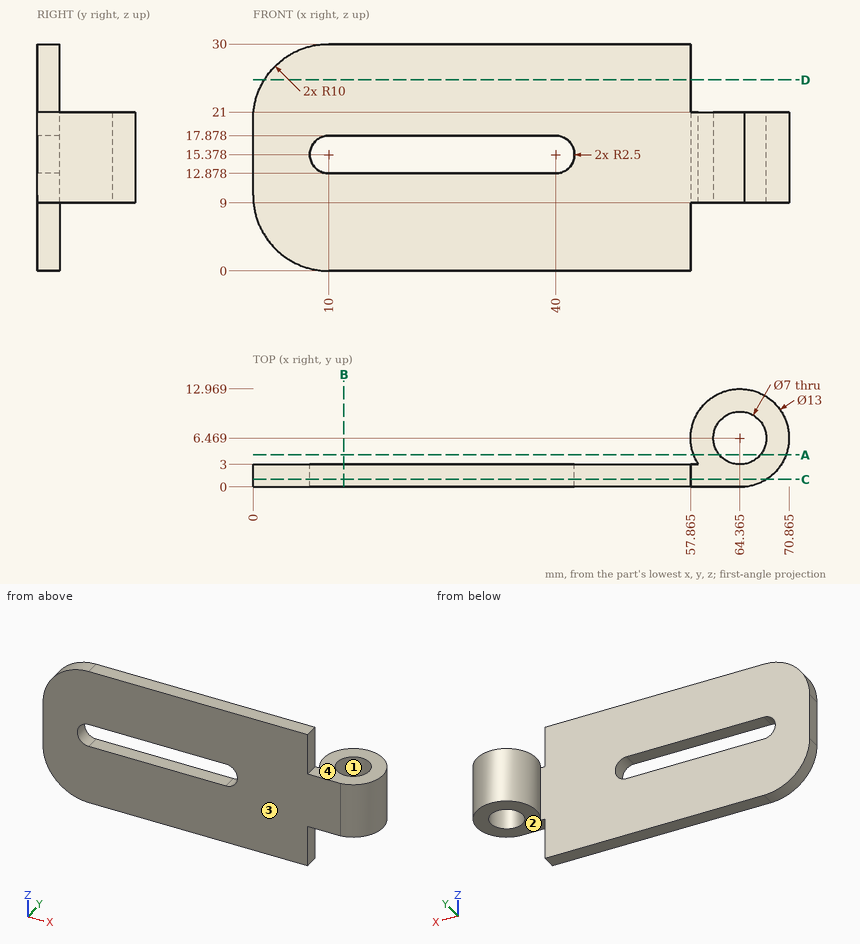
For this review, use the dimensioned drawing (mm, ordinates from the lowest corner) and the shaded views. A direction names the side the tool comes from. Round coordinates to 2 decimals unless told otherwise and drop trailing zeros. Loops run counter-clockwise (first coordinate to the right, second up) from the corner with the lowest first, then second, coordinate; pieces in that order, holes last. Notation, with made-up numbers: (62, 59.25) -> (120, 59.25) arc R25 cw to (120, 93.25) -> close; hole circle Ø8 at (3, 26.25). An arc over 180 degrees is marked (long way). Write item = value, one per line. Start each with the question number.
Item 1: To check wall thickness, follow L1, parallel to Z at x = 26, y = 2; L2, parallel to Y at x = 42, z = 12.5; L3, parallel to X at y = 7.25, z = 10.5 (1 decimal). State the ranges of each line that lie inside material, in increasing order.
Item 2: For the marked faces 3 and 4, list the 3-axis set-ups (+Z, -Z, +X, -X, +Y, -Y) from which the entire face can be reached by the end or side of a thin tool; tool diameter is ignored.
Item 3: Insertion check: pin 1 (2.5 mm diameter, centred on y = 1.5, z = 4, fed in from +X) (1 decimal); pin 2 (6.5 mm diameter, centred on x = 64.5, y = 5, fed in from +Z); pin 3 (6 mm diameter, centred on y = 4.5, z = 23.5, fed in from -X). Each pin has a flat end and moves straight along its axis. Give the tip position at first contact, or say it passes through.
Item 4: Take a section at A-A on y = 4.25. Give the boundary of the cut face in (x, z) (1 decimal).
Item 5: Mouldability with a two-part tool opening along X and no side actions: class the marked faces 1 and 2 as released by +X, released by -X, zero draft, split by the parting line, or undercut.
Item 6: Take a section at D-D on z = 25.25. Give the boundary of the cut face in (x, y) (1 decimal).
Item 7: Take a section at B-B on x = 12. Give the boundary of the cut face in (y, z).
Item 8: Take a section at C-C on y = 1. Give the boundary of the cut face in (x, z) (1 decimal), plus the area to 3 significant figures.
Result:
q1.L1 = 0 to 12.88, 17.88 to 30
q1.L2 = 0 to 3
q1.L3 = 57.9 to 61, 67.8 to 70.8
q2.face_3 = +Z, -Z, +X, -X, -Y
q2.face_4 = +Z, +X, +Y, -Y
q3.pin_1 = 57.9
q3.pin_2 = 21
q3.pin_3 = 0.04
q4.outline = (58.3, 9) -> (61.7, 9) -> (61.7, 21) -> (58.3, 21) -> close; (67.1, 9) -> (70.5, 9) -> (70.5, 21) -> (67.1, 21) -> close
q5.face_1 = undercut
q5.face_2 = zero draft
q6.outline = (1.5, 0) -> (57.9, 0) -> (57.9, 3) -> (1.5, 3) -> close
q7.outline = (0, 0) -> (3, 0) -> (3, 12.88) -> (0, 12.88) -> close; (0, 17.88) -> (3, 17.88) -> (3, 30) -> (0, 30) -> close
q8.outline = (0, 10) arc R10 ccw to (10, 0) -> (57.9, 0) -> (57.9, 9) -> (67.9, 9) -> (67.9, 21) -> (57.9, 21) -> (57.9, 30) -> (10, 30) arc R10 ccw to (0, 20) -> close; hole (10, 12.9) -> (40, 12.9) arc R2.5 ccw to (40, 17.9) -> (10, 17.9) arc R2.5 ccw to start
q8.area = 1,640 mm²
